```python
from build123d import *

# Parameters (mm, degrees)
EXTRUDE_1_DEPTH        = 20
SKETCH_3_R             = 5
EXTRUDE_2_DEPTH        = 80
SKETCH_4_OUTSIDE_W     = 56.366
SKETCH_4_OUTSIDE_H     = 88.366
SKETCH_4_OUTSIDE_W_2   = 11.216089963
SKETCH_4_OUTSIDE_H_2   = 6
CUT_EXTRUDE_1_DEPTH    = 10
HOLE_WIZARD_M4_1_D     = 3.3
HOLE_WIZARD_M4_1_DEPTH = 10.1
HOLE_WIZARD_M4_1_TIP   = 0.991420021


with BuildPart() as part:
    # 草图2 → 凸台-拉伸1 (new body)
    with BuildSketch(Plane.XY):
        with BuildLine():
            Line((2.343208281, 0.995863519), (40, 17))
            Line((40, 17), (45, 17))
            ThreePointArc((45, 17), (53.838834765, 20.661165235), (57.5, 29.5))
            Line((57.5, 29.5), (57.5, 42))
            Line((57.5, 42), (62.5, 42))
            Line((62.5, 42), (62.5, -10))
            Line((62.5, -10), (57.5, -10))
            Line((57.5, -10), (40, -10))
            Line((40, -10), (-20.046049724, -10))
            Line((-20.046049724, -10), (-20.046049724, 0))
            Line((-20.046049724, 0), (-20.046049724, 25))
            Line((-20.046049724, 25), (-15.046049724, 25))
            Line((-15.046049724, 25), (-15.046049724, 12.5))
            ThreePointArc((-15.046049724, 12.5), (-9.442943044, 2.074892685), (2.343208281, 0.995863519))
        make_face()
    extrude(amount=EXTRUDE_1_DEPTH)

    # 草图3 → 凸台-拉伸2 (add)
    with BuildSketch(Plane.ZY.offset(20.046049724)):
        with Locations(Location((10, 0, 0), (0, 0, 180))):
            Circle(SKETCH_3_R)
    extrude(amount=EXTRUDE_2_DEPTH)

    # 草图4 outside → 切除-拉伸1 (cut)
    with BuildSketch(Plane.ZY.offset(100.046049724)):
        with Locations((10, 16)):
            Rectangle(SKETCH_4_OUTSIDE_W, SKETCH_4_OUTSIDE_H)
        with Locations((9.391955019, 0)):
            Rectangle(SKETCH_4_OUTSIDE_W_2, SKETCH_4_OUTSIDE_H_2, mode=Mode.SUBTRACT)
    extrude(amount=-CUT_EXTRUDE_1_DEPTH, mode=Mode.SUBTRACT)

    # M4 螺纹孔1
    with Locations(Plane(origin=(0, 3, 0), x_dir=(1, 0, 0), z_dir=(0, 1, 0))):
        with Locations((-95.046049724, -10)):
            Hole(HOLE_WIZARD_M4_1_D / 2, depth=HOLE_WIZARD_M4_1_DEPTH)
            with Locations((0, 0, -(HOLE_WIZARD_M4_1_DEPTH + HOLE_WIZARD_M4_1_TIP / 2))):  # 118° drill point
                Cone(0, HOLE_WIZARD_M4_1_D / 2, HOLE_WIZARD_M4_1_TIP, mode=Mode.SUBTRACT)


solid = part.part
```
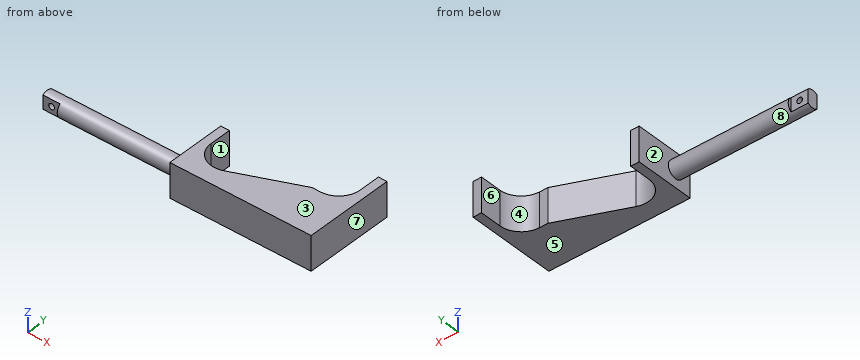
Part model, mm, in its own coordinate system. Face numbers are marked on the shaded views. A direction names the side the tool comes from. Give positions to 0.01 mm unless a question says otherwise; leave off trailing zeros. Order: outer loops, then holes, each group sorted by start corner. A loop starts at its lowest first (then second) coordinate and runs counter-clockwise, first axis right, second up. Notation, with made-up numbers: M 11,-5 L 44,-5 A26 ccw 44,23 Z; hole C 3,32.5 d5. An arc over 180 degrees is marked long. Use a Markdown table: item, result. Add a question column.
(1) Probe line 1 along X through (y, z) = (23.5, 10.5); line 2 along X through (y, z) = (-0.25, 10); line 3 along X through (y, z) = (29, 7). List the from-to ranges inside material, lowest first. Write a range as [from, to].
(2) Mould opens along X. For the marked faces 1, 2 and 3 say: +X half, -X half, draft (parallel to the pull), parting line (faces both ways), or undercut.
(3) Saw through at C-C, the plane x = -17. Give the cut face in (y, z), and give its area (3 significant figures).
(4) Saw through at D-D, the plane y = 34. Give the cut face in (x, z), and give its area (3 significant figures).
(5) Drop flat-ended pins along their axis: P1, Ø1.6, axis at y = 4.5, z = 11.5, coming from the -X side; P2, Ø5, axis at x = -73.5, z = 3, coming from the +Y side; P3, Ø1.5, axis at x = -18, z = 9.5, coming from the +Y side. Give the stop position or say it passes through.
(6) Saw through at B-B, the plane y = 9.5. Give the cut face in (x, z).
(7) 3-axis set-ups, long thin cutter, end or side, ignore diameter. For the marked faces 4, 5, 6, 7 and 8: which of +Z, -Z, +X, -X, +Y, -Y reach the whole face in a straight line?
(8) Saw through at A-A, the plane z = 10. Give the cut face in (x, y), and give its area (3 significant figures).
Answer key:
| question | item | result |
|---|---|---|
| 1 | line 1 | [-20.05, -15.05], [55.97, 62.5] |
| 1 | line 2 | [-100.05, -96.7], [-93.4, 62.5] |
| 1 | line 3 | [57.49, 62.5] |
| 2 | face 1 | undercut |
| 2 | face 2 | -X half |
| 2 | face 3 | draft |
| 3 | outline | M -10,0 L 25,0 L 25,20 L -10,20 Z |
| 3 | area | 700 mm^2 |
| 4 | outline | M 57.5,0 L 62.5,0 L 62.5,20 L 57.5,20 Z |
| 4 | area | 100 mm^2 |
| 5 | P1 | x = -90.05 |
| 5 | P2 | y = 2.18 |
| 5 | P3 | y = 25 |
| 6 | outline | M -20.05,0 L -14.68,0 L -14.68,20 L -20.05,20 Z; M 22.35,0 L 62.5,0 L 62.5,20 L 22.35,20 Z |
| 7 | face 4 | +Z, -Z, +Y |
| 7 | face 5 | -Z, +X, -X, +Y, -Y |
| 7 | face 6 | +Z, -Z, -X, +Y |
| 7 | face 7 | +Z, -Z, +X, +Y, -Y |
| 7 | face 8 | -X |
| 8 | outline | M -100.05,-3 L -96.7,-3 L -96.7,3 L -100.05,3 Z; M -93.4,-3 L -90.05,-3 L -90.05,-5 L -20.05,-5 L -20.05,-10 L 62.5,-10 L 62.5,42 L 57.5,42 L 57.5,29.5 A12.5 cw 45,17 L 40,17 L 2.34,1 A12.5 cw -15.05,12.5 L -15.05,25 L -20.05,25 L -20.05,5 L -90.05,5 L -90.05,3 L -93.4,3 Z |
| 8 | area | 2,610 mm^2 |
